```python
from build123d import *

# Parameters (mm, degrees)
SKETCH1_W                                            = 40
SKETCH1_H                                            = 20
BOSS_EXTRUDE1_DEPTH                                  = 25
SKETCH2_W                                            = 60
SKETCH2_H                                            = 70
BOSS_EXTRUDE2_DEPTH                                  = 8
CUT_EXTRUDE1_DEPTH                                   = 62.02458521
CHAMFER1_SIZE                                        = 10
HOLE_SIZE_PER_SOCKET_HEAD_CAP_SCREW_TYPE_D           = 4.5
HOLE_SIZE_PER_SOCKET_HEAD_CAP_SCREW_TYPE_CBORE_D     = 8
HOLE_SIZE_PER_SOCKET_HEAD_CAP_SCREW_TYPE_CBORE_DEPTH = 4.6
HOLE_SIZE_PER_SOCKET_HEAD_CAP_SCREW_2_D              = 4.5
HOLE_SIZE_PER_SOCKET_HEAD_CAP_SCREW_2_CBORE_D        = 8
HOLE_SIZE_PER_SOCKET_HEAD_CAP_SCREW_2_CBORE_DEPTH    = 4.6
M5_TAPPED_HOLE1_D                                    = 4.2
M5_TAPPED_HOLE1_DEPTH                                = 12.4
M5_TAPPED_HOLE1_TIP                                  = 1.2618073
M3_TAPPED_HOLE1_D                                    = 2.5
M3_TAPPED_HOLE1_DEPTH                                = 7.5
M3_TAPPED_HOLE1_TIP                                  = 0.751075774


with BuildPart() as part:
    # Sketch1 → Boss-Extrude1 (new, symmetric)
    with BuildSketch(Plane.XY):
        Rectangle(SKETCH1_W, SKETCH1_H)
    extrude(amount=BOSS_EXTRUDE1_DEPTH, both=True)

    # Sketch2 → Boss-Extrude2 (add)
    with BuildSketch(Plane.XZ.offset(10)):
        with Locations((0, 10)):
            Rectangle(SKETCH2_W, SKETCH2_H)
    extrude(amount=BOSS_EXTRUDE2_DEPTH)

    # Sketch3 → Cut-Extrude1 (cut, through all)
    with BuildSketch(Plane.XY.offset(25)):
        with BuildLine():
            Line((-7.5, 10), (-11.541451884, 3))
            ThreePointArc((-11.541451884, 3), (-11.541451884, 1), (-9.809401077, 0))
            Line((-9.809401077, 0), (9.809401077, 0))
            ThreePointArc((9.809401077, 0), (11.541451884, 1), (11.541451884, 3))
            Line((11.541451884, 3), (7.5, 10))
            Line((7.5, 10), (-7.5, 10))
        make_face()
    extrude(amount=-CUT_EXTRUDE1_DEPTH, mode=Mode.SUBTRACT)

    # Chamfer1
    chamfer1_edges = [part.edges().sort_by_distance(p)[0] for p in [
        (-30, -14, 45),
        (30, -14, 45),
    ]]
    chamfer(chamfer1_edges, length=CHAMFER1_SIZE)

    # Hole Size per Socket Head Cap Screw Type (through all)
    with Locations(Plane.XZ.offset(18)):
        with Locations((7, 40), (-7, 40)):
            CounterBoreHole(HOLE_SIZE_PER_SOCKET_HEAD_CAP_SCREW_TYPE_D / 2, HOLE_SIZE_PER_SOCKET_HEAD_CAP_SCREW_TYPE_CBORE_D / 2, HOLE_SIZE_PER_SOCKET_HEAD_CAP_SCREW_TYPE_CBORE_DEPTH)

    # Hole Size per Socket Head Cap Screw  2 (through all)
    with Locations(Plane(origin=(0, -10, 0), x_dir=(-1, 0, 0), z_dir=(0, 1, 0))):
        with Locations((25, -17.5), (25, 7.5), (-25, -17.5), (-25, 7.5)):
            CounterBoreHole(HOLE_SIZE_PER_SOCKET_HEAD_CAP_SCREW_2_D / 2, HOLE_SIZE_PER_SOCKET_HEAD_CAP_SCREW_2_CBORE_D / 2, HOLE_SIZE_PER_SOCKET_HEAD_CAP_SCREW_2_CBORE_DEPTH)

    # M5 Tapped Hole1
    with Locations(Plane(origin=(20, 0, 0), x_dir=(0, 0, -1), z_dir=(1, 0, 0))):
        with Locations((-3, 2.5)):
            Hole(M5_TAPPED_HOLE1_D / 2, depth=M5_TAPPED_HOLE1_DEPTH)
            with Locations((0, 0, -(M5_TAPPED_HOLE1_DEPTH + M5_TAPPED_HOLE1_TIP / 2))):  # 118° drill point
                Cone(0, M5_TAPPED_HOLE1_D / 2, M5_TAPPED_HOLE1_TIP, mode=Mode.SUBTRACT)

    # M3 Tapped Hole1
    with Locations(Plane(origin=(0, 0, -25), x_dir=(-1, 0, 0), z_dir=(0, 0, -1))):
        with Locations((14, 5), (-14, 5)):
            Hole(M3_TAPPED_HOLE1_D / 2, depth=M3_TAPPED_HOLE1_DEPTH)
            with Locations((0, 0, -(M3_TAPPED_HOLE1_DEPTH + M3_TAPPED_HOLE1_TIP / 2))):  # 118° drill point
                Cone(0, M3_TAPPED_HOLE1_D / 2, M3_TAPPED_HOLE1_TIP, mode=Mode.SUBTRACT)


solid = part.part
```
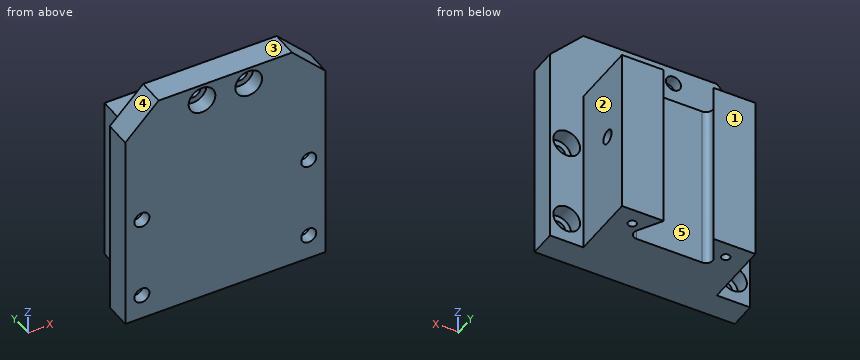
The listing builds one solid part. Answer for the finished solid, in the listing's coordinates (mm). Face numbers are marked on the shaded views. A direction names the side the tool comes from. Give positions to 0.01 mm unless a question says otherwise; leave off trailing zeros. Loops run counter-clockwise (first coordinate to the right, second up) from the corner with the lowest first, then second, coordinate; pieces in that order, holes last. Notation, with made-up numbers: M 36.5,68.25 L 50.5,68.25 A28 ccw 50.5,88.25 Z; hole C -9,-22 d3. An arc over 180 degrees is marked long. One line per item, written item: value.
Q1. A cutting plane is placed at C-C on z = 17.5. Determine the outline of the cut face in (x, y), then the cut area to 3 significant figures.
Working result:
outline: M -30,-18 L 30,-18 L 30,-10 L 20,-10 L 20,10 L 7.5,10 L 11.54,3 A2 cw 9.81,0 L -9.81,0 A2 cw -11.54,3 L -7.5,10 L -20,10 L -20,-10 L -30,-10 Z
area: 1,080 mm^2
Q2. Flat-ended cylindrical pins translate along their axes: P1, Ø1, axis at y = -4, z = -14.5, coming from the -X side; P2, Ø5, axis at x = 7, z = 40, coming from the +Y side; P3, Ø5, axis at y = -7, z = -11, coming from the +X side; P4, Ø2.5, axis at x = -25, z = 8, coming from the +Y side. Find the tip coordinate at first contact, or state that the pin passes through.
Working result:
P1: stops at x = -20
P2: stops at y = -10
P3: stops at x = 20
P4: passes through
Q3. For the marked faces 1 and 2, determine the directions among +Z, -Z, +X, -X, +Y, -Y from which every point of the face is accessible in a straight line to the end or side of a thin tool.
Working result:
face 1: +Z, -Z, +X, -X, +Y
face 2: +Z, -Z, +X, +Y
Q4. Find the intervals of material crossed by line 1 (Z direction, x = -25, y = -12.9); line 2 (X direction, y = -10.25, z = 6); line 3 (Y direction, x = -14, z = -20.5), in increasing order. Write a range as from..to.
Working result:
line 1: z = -25..-21.5, -13.5..3.5, 11.5..40
line 2: x = -30..-28.71, -21.29..21.29, 28.71..30
line 3: y = -18..3.75, 6.25..10
Q5. A cutting plane is placed at D-D on z = 7.5. Give the number of separate pieces and of enclosed holes in the cut face, then the cut area to 3 significant figures.
Working result:
separate pieces: 3
enclosed holes: 0
area: 974 mm^2
Q6. A cutting plane is placed at B-B on z = 40. Determine the outline of the cut face in (x, y), then the cut area to 3 significant figures.
Working result:
outline: M -25,-18 L -11,-18 L -11,-13.4 L -9.25,-13.4 L -9.25,-10 L -25,-10 Z; M -4.75,-13.4 L -3,-13.4 L -3,-18 L 3,-18 L 3,-13.4 L 4.75,-13.4 L 4.75,-10 L -4.75,-10 Z; M 9.25,-13.4 L 11,-13.4 L 11,-18 L 25,-18 L 25,-10 L 9.25,-10 Z
area: 296 mm^2
Q7. A cutting plane is placed at A-A on x = 25. Determine the outline of the cut face in (y, z).
Working result:
outline: M -18,-25 L -10,-25 L -10,-21.5 L -14.6,-21.5 L -14.6,-19.75 L -18,-19.75 Z; M -18,-15.25 L -14.6,-15.25 L -14.6,-13.5 L -10,-13.5 L -10,3.5 L -14.6,3.5 L -14.6,5.25 L -18,5.25 Z; M -18,9.75 L -14.6,9.75 L -14.6,11.5 L -10,11.5 L -10,40 L -18,40 Z
Q8. Determine the mould class of the marked faces 3, 4 and 5 for opening direction X: +X half, -X half, draft (parallel to the pull), parting line (faces both ways), or undercut.
Working result:
face 3: draft
face 4: -X half
face 5: undercut
